Read the model definition and answer for the solid it produces. Units are mm, in the model's axes. A direction names the side the tool comes from. Round coordinates to 2 decimals unless told otherwise and drop trailing zeros. Write each loop counter-clockwise with the first axis right and the second up, starting at its lowest first coordinate (ties: lowest second). Pieces come first, ordered by that corner, then holes. Notation, with made-up numbers: (82.5, 53.5) -> (97.5, 53.5) arc R24 cw to (97.5, 87.5) -> close; hole circle Ø4 at (-8.75, 34.5). An arc over 180 degrees is marked (long way). Return JSON: item names as keys, results as strings. Group by question number.
(1) Given pin 1 (1.8 mm diameter, centred on y = -14, z = 3.5, fed in from -X); pin 2 (2 mm diameter, centred on x = 148, z = 4.5, fed in from -Y); pin 3 (1 mm diameter, centred on y = 61, z = 1.5, fed in from -X), each flat-ended and moving along its own axis, determine where each tip first touches the part or whether it passes through.
(2) A cutting plane is placed at D-D on x = 139.5. Give the vertices of the cut face in (y, z).
(3) A cutting plane is placed at C-C on y = 53. Give the vertices of the cut face in (x, z), then the cut area to 3 significant figures.
(4) A cutting plane is placed at B-B on z = 3.1. Give the vertices of the cut face in (x, y), then the cut area to 3 significant figures.
(5) Straight lines are drawn through the part: line 1 (X direction, y = 48, z = 2.15); line 2 (Y direction, x = 139, z = 4.3); line 3 (X direction, y = 72, z = 3.3). For each, find the intervals that lie inside material, in ascending order.
(6) A cutting plane is placed at A-A on y = 85. Give the vertices of the cut face in (x, z).
(7) For faces 1 (the flat face through (126.528, -15, 3)), 2 (the flat face through (130, 37, 0)), 3 (the flat face through (136.029, 53, 3)), determine the directions among +Z, -Z, +X, -X, +Y, -Y from which every point of the face is accessible in a straight line to the end or side of a thin tool.
(8) The mould has two halves that part along X. Classify faces 4 (the flat face through (151.529, -15, 3)), 5 (the flat face through (130, 37, 6)): released by +X, released by -X, zero draft, split by the parting line, or undercut.
```python
from build123d import *

# Parameters (mm, degrees)
BOSS_EXTRUDE1_DEPTH = 6
SKETCH2_W           = 6
SKETCH2_H           = 59.975118876
CUT_EXTRUDE1_DEPTH  = 6


with BuildPart() as part:
    # Sketch1 → Boss-Extrude1 (new body)
    with BuildSketch(Plane.XY):
        Polygon((106.551616656, -20.563894675), (102.587015051, 90.196105325), (122.52424687, 90.909749071), (122.810419801, 82.914869143), (147.794419574, 83.809159551), (147.508246643, 91.804039479), (167.445478462, 92.517683224), (171.410080068, -18.242316776), (151.529151094, -18.953945188), (151.529151094, -10.563897816), (126.528434018, -10.563897816), (126.528434018, -19.848833984), align=None)
    extrude(amount=BOSS_EXTRUDE1_DEPTH)

    # Sketch2 → Cut-Extrude1 (cut)
    with BuildSketch(Plane.XY.offset(6)):
        with Locations((139.028792556, 53.898004923)):
            Rectangle(SKETCH2_W, SKETCH2_H)
    extrude(amount=-CUT_EXTRUDE1_DEPTH, mode=Mode.SUBTRACT)


solid = part.part
```
Checks:
{
 "1": {"pin 1": "stops at x = 106.28", "pin 2": "stops at y = -10.56", "pin 3": "stops at x = 103.61"},
 "2": {"outline": "(-10.56, 0) -> (23.91, 0) -> (23.91, 6) -> (-10.56, 6) -> close"},
 "3": {"outline": "(103.92, 0) -> (136.03, 0) -> (136.03, 6) -> (103.92, 6) -> close; (142.03, 0) -> (168.86, 0) -> (168.86, 6) -> (142.03, 6) -> close", "area": "354 mm^2"},
 "4": {"outline": "(102.59, 90.2) -> (106.55, -20.56) -> (126.53, -19.85) -> (126.53, -10.56) -> (151.53, -10.56) -> (151.53, -18.95) -> (171.41, -18.24) -> (167.45, 92.52) -> (147.51, 91.8) -> (147.79, 83.81) -> (142.03, 83.6) -> (142.03, 23.91) -> (136.03, 23.91) -> (136.03, 83.39) -> (122.81, 82.91) -> (122.52, 90.91) -> close", "area": "6,410 mm^2"},
 "5": {"line 1": "x = 104.1 to 136.03, 142.03 to 169.04", "line 2": "y = -10.56 to 23.91", "line 3": "x = 103.24 to 136.03, 142.03 to 168.18"},
 "6": {"outline": "(102.77, 0) -> (122.74, 0) -> (122.74, 6) -> (102.77, 6) -> close; (147.75, 0) -> (167.71, 0) -> (167.71, 6) -> (147.75, 6) -> close"},
 "7": {"face 1": "+Z, -Z, -Y", "face 2": "-Z, +X, -X, +Y, -Y", "face 3": "+Z, -Z, +Y"},
 "8": {"face 4": "undercut", "face 5": "zero draft"}
}
